Source: CAD feature listing. Evaluate the final solid. Frame: model axes, mm. A direction names the side the tool comes from. Round coordinates to 2 decimals unless told otherwise and drop trailing zeros. Write each loop counter-clockwise with the first axis right and the second up, starting at its lowest first coordinate (ties: lowest second). Pieces come first, ordered by that corner, then holes.
from build123d import *

# Parameters (mm, degrees)
SKETCH1_R                                           = 45
SKETCH1_R_2                                         = 27
BOSS_EXTRUDE1_DEPTH                                 = 13
SKETCH2_R                                           = 80
BOSS_EXTRUDE2_DEPTH                                 = 10
CUT_EXTRUDE1_DEPTH                                  = 114.881517377
CIRPATTERN1_COUNT                                   = 4
SKETCH6_R                                           = 27
CUT_EXTRUDE2_DEPTH                                  = 114.881517377
CBORE_FOR_M8_HEX_SOCKET_HEAD_CAP_SCREW1_D           = 9
CBORE_FOR_M8_HEX_SOCKET_HEAD_CAP_SCREW1_CBORE_D     = 15
CBORE_FOR_M8_HEX_SOCKET_HEAD_CAP_SCREW1_CBORE_DEPTH = 8.6
CIRPATTERN2_COUNT                                   = 8


with BuildPart() as part:
    # Sketch1 → Boss-Extrude1 (new body)
    with BuildSketch(Plane.XY):
        with Locations(Location((0, 0, 0), (0, 0, 180))):
            Circle(SKETCH1_R)
        with Locations(Location((0, 0, 0), (0, 0, 180))):
            Circle(SKETCH1_R_2, mode=Mode.SUBTRACT)
    extrude(amount=BOSS_EXTRUDE1_DEPTH)

    # Sketch2 → Boss-Extrude2 (add)
    with BuildSketch(Plane.XY):
        Circle(SKETCH2_R)
    extrude(amount=-BOSS_EXTRUDE2_DEPTH)

    # Sketch3 → M8 Tapped Hole1 (revolve, cut)
    with BuildSketch(Plane(origin=(0, -57, 0), x_dir=(0, -1, 0), z_dir=(1, 0, 0))):
        Polygon((0, 0), (0, 24.342926105), (3.4, 22.3), (3.4, 0), align=None)
    m8_tapped_hole1 = revolve(axis=Axis((0, -57, 6.35), (0, 0, -1)), mode=Mode.SUBTRACT)

    # Sketch5 → Cut-Extrude1 (cut, through all)
    with BuildSketch(Plane.XY):
        with BuildLine():
            Line((45, 49.271909465), (55, 49.271909465))
            ThreePointArc((55, 49.271909465), (59.271909465, 45), (55, 40.728090535))
            Line((55, 40.728090535), (45, 40.728090535))
            ThreePointArc((45, 40.728090535), (40.728090535, 45), (45, 49.271909465))
        make_face()
        with BuildLine():
            Line((45, -40.728090535), (55, -40.728090535))
            ThreePointArc((55, -40.728090535), (59.271909465, -45), (55, -49.271909465))
            Line((55, -49.271909465), (45, -49.271909465))
            ThreePointArc((45, -49.271909465), (40.728090535, -45), (45, -40.728090535))
        make_face()
        with BuildLine():
            Line((-45, -40.728090535), (-55, -40.728090535))
            ThreePointArc((-55, -40.728090535), (-59.271909465, -45), (-55, -49.271909465))
            Line((-55, -49.271909465), (-45, -49.271909465))
            ThreePointArc((-45, -49.271909465), (-40.728090535, -45), (-45, -40.728090535))
        make_face()
        with BuildLine():
            Line((-45, 49.271909465), (-55, 49.271909465))
            ThreePointArc((-55, 49.271909465), (-59.271909465, 45), (-55, 40.728090535))
            Line((-55, 40.728090535), (-45, 40.728090535))
            ThreePointArc((-45, 40.728090535), (-40.728090535, 45), (-45, 49.271909465))
        make_face()
    extrude(amount=-CUT_EXTRUDE1_DEPTH, mode=Mode.SUBTRACT)

    # CirPattern1: M8 Tapped Hole1 ×4 about axis
    cirpattern1_axis = Axis((0, 0, 0), (0, 0, 1))
    for i in range(1, CIRPATTERN1_COUNT):
        add(m8_tapped_hole1.rotate(cirpattern1_axis, i * 360 / CIRPATTERN1_COUNT), mode=Mode.SUBTRACT)

    # Sketch6 → Cut-Extrude2 (cut, through all)
    with BuildSketch(Plane.XY):
        with Locations(Location((0, 0, 0), (0, 0, 180))):
            Circle(SKETCH6_R)
    extrude(amount=-CUT_EXTRUDE2_DEPTH, mode=Mode.SUBTRACT)

    # CBORE for M8 Hex Socket Head Cap Screw1 (through all)
    with Locations(Plane(origin=(0, 0, -10), x_dir=(-1, 0, 0), z_dir=(0, 0, -1))):
        with Locations((35, 0)):
            cbore_for_m8_hex_socket_head_cap_screw1 = CounterBoreHole(CBORE_FOR_M8_HEX_SOCKET_HEAD_CAP_SCREW1_D / 2, CBORE_FOR_M8_HEX_SOCKET_HEAD_CAP_SCREW1_CBORE_D / 2, CBORE_FOR_M8_HEX_SOCKET_HEAD_CAP_SCREW1_CBORE_DEPTH)

    # CirPattern2: CBORE for M8 Hex Socket Head Cap Screw1 ×8 about axis
    cirpattern2_axis = Axis((0, 0, 0), (0, 0, 1))
    for i in range(1, CIRPATTERN2_COUNT):
        add(cbore_for_m8_hex_socket_head_cap_screw1.rotate(cirpattern2_axis, i * 360 / CIRPATTERN2_COUNT), mode=Mode.SUBTRACT)


solid = part.part
1) Section query A-A on x = 35. Return the cut outline in (y, z), then the cut area to 3 significant figures.
Taken from the geometry:
outline: (-71.94, -10) - (-7.5, -10) - (-7.5, -1.4) - (-4.5, -1.4) - (-4.5, 13) - (-28.28, 13) - (-28.28, 0) - (-71.94, 0) - close; (4.5, -1.4) - (7.5, -1.4) - (7.5, -10) - (71.94, -10) - (71.94, 0) - (28.28, 0) - (28.28, 13) - (4.5, 13) - close
area: 1,920 mm2
2) Section query C-C on z = -4.75. State how many separate pieces and enclosed holes the cut face has, then the cut area to 3 significant figures.
Taken from the geometry:
separate pieces: 1
enclosed holes: 17
area: 15,700 mm2
3) Reachability of faces 1 (the face through (-29.317, -18.8, -5.76)), 2 (the face through (50, -49.272, -5)) from +Z, -Z, +X, -X, +Y, -Y: full face, straight path, thin tool, end or side. Return the list, or none.
Taken from the geometry:
face 1: -Z
face 2: +Z, -Z
4) Material intervals for line 1 (X direction, y = 0.5, z = 9.5); line 2 (Y direction, x = -44.5, z = -3.75); line 3 (X direction, y = 5.5, z = -6), sorted ascending.
Taken from the geometry:
line 1: x = -45 to -39.47, -30.53 to -27, 27 to 30.53, 39.47 to 45
line 2: y = -66.48 to -49.24, -40.76 to 40.76, 49.24 to 66.48
line 3: x = -79.81 to -40.1, -29.9 to -26.43, 26.43 to 29.9, 40.1 to 79.81
5) Contact query for flat-ended pins moving along their axis: P1, Ø10.5, axis at x = 0, y = 35, coming from the -Z side; P2, Ø10, axis at x = 49.5, y = -58, coming from the +Z side; P3, Ø6, axis at x = 42, z = -6, coming from the -Y side. Output: stop coordinate, or through.
Taken from the geometry:
P1: stops at z = -1.4
P2: stops at z = 0
P3: stops at y = -69.85
6) Section query D-D on x = -57. Return the cut outline in (y, z), then the cut area to 3 significant figures.
Taken from the geometry:
outline: (-56.13, -10) - (-48.77, -10) - (-48.77, 0) - (-56.13, 0) - close; (-41.23, -10) - (-3.4, -10) - (-3.4, 0) - (-41.23, 0) - close; (3.4, -10) - (41.23, -10) - (41.23, 0) - (3.4, 0) - close; (48.77, -10) - (56.13, -10) - (56.13, 0) - (48.77, 0) - close
area: 904 mm2
